Design review of the part built by this model. Coordinates are the model's own, in mm. A direction names the side the tool comes from. Give positions to 0.01 mm unless a question says otherwise; leave off trailing zeros. Order: outer loops, then holes, each group sorted by start corner. A loop starts at its lowest first (then second) coordinate and runs counter-clockwise, first axis right, second up. Notation, with made-up numbers: (54.5, -29) -> (98.5, -29) arc R28 cw to (98.5, -7) -> close; hole circle Ø8 at (73, -39.5). An arc over 180 degrees is marked (long way). One line per item, written item: value. Start each with the question number.
1) Tool access review of faces 1 (the face through (230, 2, 120)), 2 (the face through (-4, 175, 66)), 3 (the face through (198, 99, 8)): name each direction out of +Z, -Z, +X, -X, +Y, -Y from which nothing blocks a thin tool from reaching the whole face with its end or side.
2) Consider section D-D (y = 0). State the section outline as (x, z) points, plus the area to 3 significant figures.
3) For pin 1 (18 mm diameter, centred on y = -110, z = 60, fed in from +X); pin 2 (1.5 mm diameter, centred on x = 127.5, y = 9.5, fed in from -Z); pin 3 (23 mm diameter, centred on y = 110, z = 60, fed in from -X); pin 4 (3 mm diameter, centred on y = -104, z = -21.5, fed in from +X), all flat-tipped, find the tip position at first contact; note any pin that passes through.
4) Consider section A-A (x = 160.5). State the section outline as (y, z) points.
5) Consider section C-C (x = -58.5). State the section outline as (y, z) points, plus the area to 3 significant figures.
6) Consider section B-B (z = 60). State how many separate pieces and enclosed holes the cut face has, plus the area to 3 significant figures.
7) The part is to be moulded in two halves that separate along X. For faces 4 (the face through (199.014, 119.915, 61.302)), 5 (the face through (-3, -173, 65)), 6 (the face through (-200, 98, 1)), say which applies: released by +X, released by -X, zero draft, split by the parting line, or undercut.
8) Wall thickness on line 1 along Y through (x, z) = (-199, 60); line 2 along X through (y, z) = (189.5, -19); line 3 along Y through (x, z) = (-93.5, 61): over which ranges is each line inside the solid? List them lowest first. Write a range as from..to.
from build123d import *

# Parameters (mm, degrees)
SKETCH_1_W          = 400
SKETCH_1_H          = 350
EXTRUDE_1_DEPTH     = 130
EXTRUDE_5_DEPTH     = 400
SHELL_2_T           = -2
SKETCH_3_W          = 60
SKETCH_3_H          = 350
EXTRUDE_2_DEPTH     = 10
SKETCH_8_W          = 250
SKETCH_8_H          = 200
CUT_EXTRUDE_1_DEPTH = 545.949881083
SKETCH_9_R          = 10
CUT_EXTRUDE_2_DEPTH = 614.954393374


with BuildPart() as part:
    # 草图1 → 凸台-拉伸1 (new body)
    with BuildSketch(Plane.XY):
        Rectangle(SKETCH_1_W, SKETCH_1_H)
    extrude(amount=EXTRUDE_1_DEPTH)

    # 草图7 → 凸台-拉伸5 (add)
    with BuildSketch(Plane.ZY.offset(200)):
        Polygon((0, 175), (-68.782844267, 363.979311471), (-181.270675963, 323.037089017), (0, -175), align=None)
    extrude(amount=-EXTRUDE_5_DEPTH)

    # 抽壳2
    shell_2_openings = [part.faces().sort_by_distance(p)[0] for p in [
        (0, 0, 130),
        (0, 343.508200244, -125.026760115),
    ]]
    offset(amount=SHELL_2_T, openings=shell_2_openings, kind=Kind.INTERSECTION)

    # 草图3 → 凸台-拉伸2 (add)
    with BuildSketch(Plane.XY.offset(130)):
        with Locations((-230, 0)):
            Rectangle(SKETCH_3_W, SKETCH_3_H)
        with Locations((230, 0)):
            Rectangle(SKETCH_3_W, SKETCH_3_H)
    extrude(amount=-EXTRUDE_2_DEPTH)

    # 草图8 → 切除-拉伸1 (cut, through all)
    with BuildSketch(Plane.XY.offset(130)):
        Rectangle(SKETCH_8_W, SKETCH_8_H)
    extrude(amount=-CUT_EXTRUDE_1_DEPTH, mode=Mode.SUBTRACT)

    # 草图9 → 切除-拉伸2 (cut, through all)
    with BuildSketch(Plane(origin=(200, 0, 0), x_dir=(0, 0, -1), z_dir=(1, 0, 0))):
        with Locations((-60, 110)):
            Circle(SKETCH_9_R)
        with Locations((-60, -110)):
            Circle(SKETCH_9_R)
        with Locations((-60, 0)):
            Circle(SKETCH_9_R)
    extrude(amount=-CUT_EXTRUDE_2_DEPTH, mode=Mode.SUBTRACT)


solid = part.part
Checked values:
1. face 1: -Z, +X, +Y, -Y
1. face 2: +Z, +X, -X, +Y
1. face 3: none
2. outline: (-260, 120) -> (-200, 120) -> (-200, 70) -> (-198, 70) -> (-198, 130) -> (-260, 130) -> close; (-200, -63.69) -> (-125, -63.69) -> (-125, -61.57) -> (-198, -61.57) -> (-198, 50) -> (-200, 50) -> close; (125, -63.69) -> (200, -63.69) -> (200, 50) -> (198, 50) -> (198, -61.57) -> (125, -61.57) -> close; (198, 70) -> (200, 70) -> (200, 120) -> (260, 120) -> (260, 130) -> (198, 130) -> close
2. area: 2,210 mm^2
3. pin 1: passes through
3. pin 2: stops at z = -67.43
3. pin 3: stops at x = -200
3. pin 4: stops at x = 200
4. outline: (-175, 0) -> (323.04, -181.27) -> (323.72, -179.39) -> (-173, 1.4) -> (-173, 130) -> (-175, 130) -> close; (173, -1.4) -> (363.3, -70.66) -> (363.98, -68.78) -> (175, 0) -> (175, 130) -> (173, 130) -> close
5. outline: (-175, 0) -> (-100, -27.3) -> (-100, -25.17) -> (-173, 1.4) -> (-173, 130) -> (-175, 130) -> close; (100, -100.09) -> (323.04, -181.27) -> (323.72, -179.39) -> (100, -97.96) -> close; (173, -1.4) -> (363.3, -70.66) -> (363.98, -68.78) -> (175, 0) -> (175, 130) -> (173, 130) -> close
5. area: 1,560 mm^2
6. separate pieces: 6
6. enclosed holes: 0
6. area: 2,740 mm^2
7. face 4: zero draft
7. face 5: undercut
7. face 6: released by -X
8. line 1: y = -175..-120, -100..-10, 10..100, 120..175
8. line 2: x = -200..-198, 198..200
8. line 3: y = -175..-173, 173..175
